```python
from build123d import *

# Parameters (mm, degrees)
SKETCH_1_R               = 90
SKETCH_1_R_2             = 45
EXTRUDE_1_DEPTH          = 5
SKETCH_3_R               = 1.5
SKETCH_5_R               = 1.5
CUT_EXTRUDE_2_DEPTH      = 67.5
PATTERN_CIRCULAR_1_COUNT = 3


with BuildPart() as part:
    # 草图1 → 凸台-拉伸1 (new body)
    with BuildSketch(Plane.XY):
        Circle(SKETCH_1_R)
        Circle(SKETCH_1_R_2, mode=Mode.SUBTRACT)
    extrude(amount=EXTRUDE_1_DEPTH)

    # 切除-扫描1: sweep along a path in 草图2
    with BuildLine(Plane.XY.offset(5)) as sweep_1_path:
        CenterArc((0, 0), 67.5, 0, 360)
    # 草图3 → 切除-扫描1 (sweep, cut)
    with BuildSketch(Plane(origin=(0, 0, 0), x_dir=(0, 0, -1), z_dir=(1, 0, 0))):
        with Locations((-5, 67.5)):
            Circle(SKETCH_3_R)
    sweep(path=sweep_1_path.line, mode=Mode.SUBTRACT)

    # 草图5 → 切除-拉伸2 (cut)
    with BuildSketch(Plane(origin=(0, 0, 0), x_dir=(1, 0, 0), z_dir=(0, 1, 0))):
        with Locations((0, -5)):
            Circle(SKETCH_5_R)
    cut_extrude_2 = extrude(amount=CUT_EXTRUDE_2_DEPTH, mode=Mode.SUBTRACT)

    # 阵列(圆周)1: 切除-拉伸2 ×3 about axis
    pattern_circular_1_axis = Axis((0, 0, 5), (0, 0, -1))
    for i in range(1, PATTERN_CIRCULAR_1_COUNT):
        add(cut_extrude_2.rotate(pattern_circular_1_axis, i * 360 / PATTERN_CIRCULAR_1_COUNT), mode=Mode.SUBTRACT)


solid = part.part
```
Read the model definition and answer for the solid it produces. Units are mm, in the model's axes. Coordinates: 2 decimals unless noted, no trailing zeros. Loops run counter-clockwise (first coordinate to the right, second up) from the corner with the lowest first, then second, coordinate; pieces in that order, holes last. Notation, with made-up numbers: (-33.75, 47.5) - (8.25, 47.5) arc R23 cw to (8.25, 62.5) - close; hole circle Ø9 at (16, 17.25). An arc over 180 degrees is marked (long way). Answer in a Markdown table with one row per item.
1. Find section A-A, the plane z = 1.8. Write down the section's boundary in (x, y), then the cut area to 3 significant figures.
Conclusion:
| item | result |
|---|---|
| outline | circle Ø180 at (0, 0); hole circle Ø90 at (0, 0) |
| area | 19,100 mm² |
2. Straight lines are drawn through the part: line 1 (X direction, y = 17.5, z = 4.75); line 2 (Y direction, x = 0, z = 2); line 3 (X direction, y = -18, z = 1.3). For each, find the intervals that lie inside material, in ascending order.
Conclusion:
| item | result |
|---|---|
| line 1 | x = -88.28 to -66.72, -63.66 to -41.46, 41.46 to 63.66, 66.72 to 88.28 |
| line 2 | y = -90 to -45, 45 to 90 |
| line 3 | x = -88.18 to -41.24, 41.24 to 88.18 |
3. Determine the mould class of faces 1 (the face through (19, 41, 0)), 2 (the face through (41.53, -79.845, 2.465)), 3 (the face through (-48.6, -28, 3.5)) for opening direction X: +X half, -X half, draft (parallel to the pull), parting line (faces both ways), or undercut.
Conclusion:
| item | result |
|---|---|
| face 1 | draft |
| face 2 | parting line |
| face 3 | undercut |
4. Given pin 1 (2 mm diameter, centred on x = 2, z = 3, fed in from +Y); pin 2 (3 mm diameter, centred on x = 27, z = 2, fed in from -Y); pin 3 (3 mm diameter, centred on x = -27.5, z = 3.5, fed in from -Y), each flat-ended and moving along its own axis, determine where each tip first touches the part or whether it passes through.
Conclusion:
| item | result |
|---|---|
| pin 1 | stops at y = 89.99 |
| pin 2 | stops at y = -86.31 |
| pin 3 | stops at y = -86.16 |
